from build123d import *

# Parameters (mm, degrees)
SKETCH1_W           = 200
SKETCH1_H           = 180
BOSS_EXTRUDE1_DEPTH = 12
CHAMFER1_SIZE       = 10
CUT_EXTRUDE1_DEPTH  = 12


with BuildPart() as part:
    # Sketch1 → Boss-Extrude1 (new body)
    with BuildSketch(Plane.XY):
        Rectangle(SKETCH1_W, SKETCH1_H)
    extrude(amount=BOSS_EXTRUDE1_DEPTH)

    # Chamfer1
    chamfer1_edges = [part.edges().sort_by_distance(p)[0] for p in [
        (100, 90, 6),
        (-100, 90, 6),
    ]]
    chamfer(chamfer1_edges, length=CHAMFER1_SIZE)

    # Sketch2 → Cut-Extrude1 (cut)
    with BuildSketch(Plane.XY.offset(12)):
        with BuildLine():
            Line((-63.5, 71), (-63.5, 59))
            ThreePointArc((-63.5, 59), (-70, 52.5), (-76.5, 59))
            Line((-76.5, 59), (-76.5, 71))
            ThreePointArc((-76.5, 71), (-70, 77.5), (-63.5, 71))
        make_face()
        with BuildLine():
            Line((76.5, 71), (76.5, 59))
            ThreePointArc((76.5, 59), (70, 52.5), (63.5, 59))
            Line((63.5, 59), (63.5, 71))
            ThreePointArc((63.5, 71), (70, 77.5), (76.5, 71))
        make_face()
    extrude(amount=-CUT_EXTRUDE1_DEPTH, mode=Mode.SUBTRACT)


solid = part.part
Input: part model. Units: mm. Frame: model coordinates. A direction names the side the tool comes from. Round coordinates to 2 decimals unless told otherwise and drop trailing zeros. Order: outer loops, then holes, each group sorted by start corner. A loop starts at its lowest first (then second) coordinate and runs counter-clockwise, first axis right, second up. Notation, with made-up numbers: (83.25, -6) - (113.25, -6) arc R26 ccw to (113.25, 21) - close; hole circle Ø8 at (2, 61.25). An arc over 180 degrees is marked (long way). Answer as a JSON object with one key per item and string values. Group by question number.
(1) Cut plane A-A (x = -70). Return loops of the section in (y, z).
(2) Cut plane C-C (y = 55). Return loops of the section in (x, z), then the cut area to 3 significant figures.
(3) Draft query along Y for faces 3 (the face through (63.5, 65, 6)), 4 (the face through (-95, 85, 6)), 5 (the face through (-70.1, 77.5, 6.1)), 6 (the face through (-100, -6, 6)). Return one class per face: released by +Y, released by -Y, zero draft, split by the parting line, or undercut.
(4) Reachability of faces 1 (the face through (-1, 90, 6)), 2 (the face through (76.5, 65, 6)) from +Z, -Z, +X, -X, +Y, -Y: full face, straight path, thin tool, end or side. Return the list, or none.
(5) Pin query (flat end, axial travel): P1, Ø4, axis at x = -72.5, y = -37.5, coming from the -Z side. Return the tip coordinate at first contact, or that it passes through.
(6) Material intervals for probe 1 along X at (y, z) = (67, 2.5); probe 2 along Y at (x, z) = (76, 9.5); probe 3 along Y at (x, z) = (-65.5, 5.5), sorted ascending. Write a range as from..to.
(7) Cut plane B-B (z = 6.25). Return loops of the section in (x, y), then the cut area to 3 significant figures.
Here are the results:
{
 "1": {"outline": "(-90, 0) - (52.5, 0) - (52.5, 12) - (-90, 12) - close; (77.5, 0) - (90, 0) - (90, 12) - (77.5, 12) - close"},
 "2": {"outline": "(-100, 0) - (-75.12, 0) - (-75.12, 12) - (-100, 12) - close; (-64.88, 0) - (64.88, 0) - (64.88, 12) - (-64.88, 12) - close; (75.12, 0) - (100, 0) - (100, 12) - (75.12, 12) - close", "area": "2,150 mm^2"},
 "3": {"face 3": "undercut", "face 4": "released by +Y", "face 5": "undercut", "face 6": "zero draft"},
 "4": {"face 1": "+Z, -Z, +X, -X, +Y", "face 2": "+Z, -Z"},
 "5": {"P1": "stops at z = 0"},
 "6": {"probe 1": "x = -100..-76.5, -63.5..63.5, 76.5..100", "probe 2": "y = -90..56.5, 73.5..90", "probe 3": "y = -90..54.31, 75.69..90"},
 "7": {"outline": "(-100, -90) - (100, -90) - (100, 80) - (90, 90) - (-90, 90) - (-100, 80) - close; hole (-76.5, 59) arc R6.5 ccw to (-63.5, 59) - (-63.5, 71) arc R6.5 ccw to (-76.5, 71) - close; hole (63.5, 59) arc R6.5 ccw to (76.5, 59) - (76.5, 71) arc R6.5 ccw to (63.5, 71) - close", "area": "35,300 mm^2"}
}
